Part print with two shaded views. Sizes in mm from the minimum x, y, z corner. A direction names the side the tool comes from. Give positions to 0.01 mm unless a question says otherwise; leave off trailing zeros. Order: outer loops, then holes, each group sorted by start corner. A loop starts at its lowest first (then second) coordinate and runs counter-clockwise, first axis right, second up. Notation, with made-up numbers: M 20,-18.75 L 31,-18.75 A30 ccw 31,5.25 Z; hole C 6.5,50.25 d6. An arc over 180 degrees is marked long. Return JSON: item names as keys, results as strings.
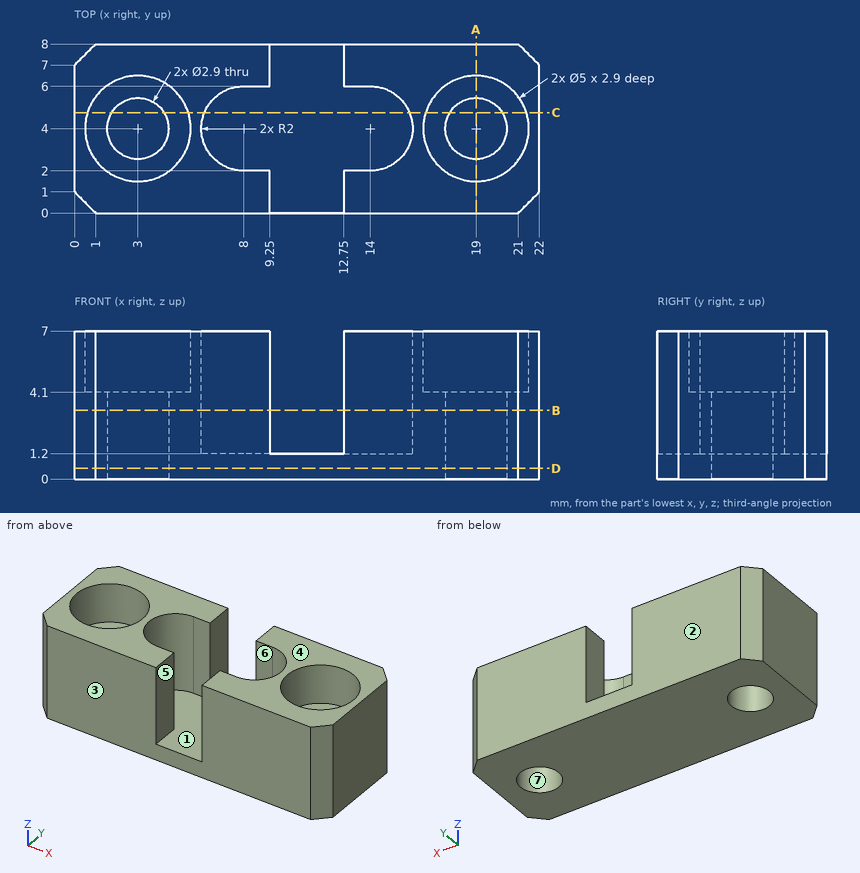
Q1. 3-axis set-ups, long thin cutter, end or side, ignore diameter. For the marked faces 5, 6 and 7: which of +Z, -Z, +X, -X, +Y, -Y reach the whole face in a straight line?
Established:
{"face 5": "+Z, +Y, -Y", "face 6": "+Z", "face 7": "+Z, -Z"}
Q2. Band-saw the part on B-B (z = 3.25). Give the cut face in (x, y), then the cut area to 3 significant figures.
Established:
{"outline": "M 0,1 L 1,0 L 9.25,0 L 9.25,2 L 8,2 A2 cw 8,6 L 9.25,6 L 9.25,8 L 1,8 L 0,7 Z; M 12.75,0 L 21,0 L 22,1 L 22,7 L 21,8 L 12.75,8 L 12.75,6 L 14,6 A2 cw 14,2 L 12.75,2 Z; hole C 3,4 d2.9; hole C 19,4 d2.9", "area": "110 mm²"}
Q3. Two-plate mould, pull along Y, no slides. Class the marked faces 1, 2, 3 and 4: +Y half, -Y half, draft (parallel to the pull), parting line (faces both ways), or undercut.
Established:
{"face 1": "undercut", "face 2": "+Y half", "face 3": "-Y half", "face 4": "draft"}
Q4. Probe line 1 along Y through (x, z) = (19, 6.4); line 2 along X through (y, z) = (5.5, 6.25); line 3 along Y through (x, z) = (13.5, 3.75). List the from-to ranges inside material, lowest first.
Established:
{"line 1": "y = 0 to 1.5, 6.5 to 8", "line 2": "x = 0 to 1, 5 to 6.68, 15.32 to 17, 21 to 22", "line 3": "y = 0 to 2, 6 to 8"}
Q5. Pin check, flat tips, straight feed: pin 1 (0.6 mm diameter, centred on y = 0.5, z = 4, fed in from -X); pin 2 (2.5 mm diameter, centred on x = 20, y = 4.5, fed in from +Z). Stop position of each tip, or through.
Established:
{"pin 1": "stops at x = 0.2", "pin 2": "stops at z = 4.1"}
Q6. Band-saw the part on D-D (z = 0.5). Give the cut face in (x, y), then the cut area to 3 significant figures.
Established:
{"outline": "M 0,1 L 1,0 L 21,0 L 22,1 L 22,7 L 21,8 L 1,8 L 0,7 Z; hole C 3,4 d2.9; hole C 19,4 d2.9", "area": "161 mm²"}
Q7. Band-saw the part on C-C (y = 4.75). Give the cut face in (x, z).
Established:
{"outline": "M 0,0 L 1.76,0 L 1.76,4.1 L 0.62,4.1 L 0.62,7 L 0,7 Z; M 4.24,0 L 17.76,0 L 17.76,4.1 L 16.62,4.1 L 16.62,7 L 15.85,7 L 15.85,1.2 L 6.15,1.2 L 6.15,7 L 5.38,7 L 5.38,4.1 L 4.24,4.1 Z; M 20.24,0 L 22,0 L 22,7 L 21.38,7 L 21.38,4.1 L 20.24,4.1 Z"}
Q8. Band-saw the part on A-A (x = 19). Give the cut face in (y, z), then the cut area to 3 significant figures.
Established:
{"outline": "M 0,0 L 2.55,0 L 2.55,4.1 L 1.5,4.1 L 1.5,7 L 0,7 Z; M 5.45,0 L 8,0 L 8,7 L 6.5,7 L 6.5,4.1 L 5.45,4.1 Z", "area": "29.6 mm²"}
